```python
from build123d import *

# Parameters (mm, degrees)
CUT_EXTRUDE1_DEPTH = 285.429253067


with BuildPart() as part:
    # Sketch1 → Revolve1 (revolve)
    with BuildSketch(Plane.XY, mode=Mode.PRIVATE) as revolve1_sk:
        Polygon((-10, 0), (-10, -30), (-200, -30), (-200, -25), (-180, -25), (-180, -5), (-200, -5), (-200, 0), align=None)
    revolve(revolve1_sk.sketch.rotate(Axis((0, 76.758624558, 0), (0, -1, 0)), 270), axis=Axis((0, 76.758624558, 0), (0, -1, 0)))

    # Sketch2 → Cut-Extrude1 (cut, through all)
    with BuildSketch(Plane(origin=(0, 0, 0), x_dir=(1, 0, 0), z_dir=(0, 1, 0))):
        with BuildLine():
            Line((-2.5, 12.682458366), (-2.5, 9.682458366))
            ThreePointArc((-2.5, 9.682458366), (0, 10), (2.5, 9.682458366))
            Line((2.5, 9.682458366), (2.5, 12.682458366))
            Line((2.5, 12.682458366), (-2.5, 12.682458366))
        make_face()
    extrude(amount=-CUT_EXTRUDE1_DEPTH, mode=Mode.SUBTRACT)


solid = part.part
```
Work out the finished part from the listing and answer in its coordinate system (mm). A direction names the side the tool comes from. Coordinates: 2 decimals unless noted, no trailing zeros. Loops run counter-clockwise (first coordinate to the right, second up) from the corner with the lowest first, then second, coordinate; pieces in that order, holes last. Notation, with made-up numbers: (-16.5, -8) - (-5.5, -8) arc R16 ccw to (-5.5, 10) - close; hole circle Ø4 at (29.25, 85). An arc over 180 degrees is marked (long way). Use a Markdown table: item, result.
Item 1: Find section C-C, the plane x = 151. Determine the outline of the cut face in (y, z).
Evaluation:
| item | result |
|---|---|
| outline | (-30, -131.14) - (-25, -131.14) - (-25, -97.97) - (-5, -97.97) - (-5, -131.14) - (0, -131.14) - (0, 131.14) - (-5, 131.14) - (-5, 97.97) - (-25, 97.97) - (-25, 131.14) - (-30, 131.14) - close |
Item 2: Find section A-A, the plane z = 0. Determine the outline of the cut face in (x, y).
Evaluation:
| item | result |
|---|---|
| outline | (-200, -30) - (-10, -30) - (-10, 0) - (-200, 0) - (-200, -5) - (-180, -5) - (-180, -25) - (-200, -25) - close; (10, -30) - (200, -30) - (200, -25) - (180, -25) - (180, -5) - (200, -5) - (200, 0) - (10, 0) - close |
Item 3: The mould has two halves that part along Z. Classify faces 1 (the cylindrical face through (0, -15, 10)), 2 (the flat face through (42, 0, -3)), 3 (the cylindrical face through (-60.075, -27.465, 190.764)): +Z half, -Z half, draft (parallel to the pull), parting line (faces both ways), or undercut.
Evaluation:
| item | result |
|---|---|
| face 1 | undercut |
| face 2 | draft |
| face 3 | parting line |
Item 4: For faces 4 (the flat face through (42, -30, 3)), 5 (the cylindrical face through (68.941, -14.86, 166.274)), determine the directions among +Z, -Z, +X, -X, +Y, -Y from which every point of the face is accessible in a straight line to the end or side of a thin tool.
Evaluation:
| item | result |
|---|---|
| face 4 | +Z, -Z, +X, -X, -Y |
| face 5 | none |
Item 5: Given pin 1 Ø1 at (y, z) = (-6.5, 103.5) entering from +X; pin 2 Ø8 at (x, y) = (114, -6.5) entering from +Z; pin 3 Ø5 at (y, z) = (-20.5, 39.5) entering from +X, each flat-ended and moving along its own axis, determine where each tip first touches the part or whether it passes through.
Evaluation:
| item | result |
|---|---|
| pin 1 | stops at x = 147.62 |
| pin 2 | stops at z = 166.84 |
| pin 3 | stops at x = 176.16 |
Item 6: Consider probe 1 along Y at (x, z) = (-112, 156.5); probe 2 along X at (y, z) = (-17.25, 0); probe 3 along X at (y, z) = (-10.5, 75). Determine where each line is inside the solid, lowest interval first. Write a range as from..to.
Evaluation:
| item | result |
|---|---|
| probe 1 | y = -30..-25, -5..0 |
| probe 2 | x = -180..-10, 10..180 |
| probe 3 | x = -163.63..163.63 |
Item 7: Find section B-B, the plane y = -17.25. Determine the outline of the cut face in (x, z).
Evaluation:
| item | result |
|---|---|
| outline | circle Ø360 at (0, 0); hole (-2.5, -12.68) - (2.5, -12.68) - (2.5, -9.68) arc R10 ccw (long way) to (-2.5, -9.68) - close |
Item 8: Find section D-D, the plane z = 43.5. Determine the outline of the cut face in (x, y).
Evaluation:
| item | result |
|---|---|
| outline | (-195.21, -30) - (195.21, -30) - (195.21, -25) - (174.66, -25) - (174.66, -5) - (195.21, -5) - (195.21, 0) - (-195.21, 0) - (-195.21, -5) - (-174.66, -5) - (-174.66, -25) - (-195.21, -25) - close |
